```python
from build123d import *

# Parameters (mm, degrees)
SKETCH1_R           = 20
SKETCH1_R_2         = 10
BOSS_EXTRUDE1_DEPTH = 8
SKETCH2_R           = 18
SKETCH2_R_2         = 13
CUT_EXTRUDE1_DEPTH  = 5.5


with BuildPart() as part:
    # Sketch1 → Boss-Extrude1 (new body)
    with BuildSketch(Plane(origin=(0, 0, 0), x_dir=(1, 0, 0), z_dir=(0, 1, 0))):
        with Locations(Location((0, 0, 0), (0, 0, 270))):
            Circle(SKETCH1_R)
        with Locations(Location((0, 0, 0), (0, 0, 270))):
            Circle(SKETCH1_R_2, mode=Mode.SUBTRACT)
    extrude(amount=BOSS_EXTRUDE1_DEPTH)

    # Sketch2 → Cut-Extrude1 (cut)
    with BuildSketch(Plane(origin=(0, 8, 0), x_dir=(1, 0, 0), z_dir=(0, 1, 0))):
        with Locations(Location((0, 0, 0), (0, 0, 270))):
            Circle(SKETCH2_R)
        with Locations(Location((0, 0, 0), (0, 0, 270))):
            Circle(SKETCH2_R_2, mode=Mode.SUBTRACT)
    extrude(amount=-CUT_EXTRUDE1_DEPTH, mode=Mode.SUBTRACT)


solid = part.part
```
Check sheet for the modelled part. Datum: model origin and axes. Units: mm. A direction names the side the tool comes from. Give positions to 0.01 mm unless a question says otherwise; leave off trailing zeros. Order: outer loops, then holes, each group sorted by start corner. A loop starts at its lowest first (then second) coordinate and runs counter-clockwise, first axis right, second up. Notation, with made-up numbers: (40, 57.5) -> (55, 57.5) arc R16 cw to (55, 65.5) -> close; hole circle Ø8 at (74, 19.5). An arc over 180 degrees is marked (long way). Use CSV: the item, a comma, the result in double quotes. Start each with the question number.
1) Material ranges on line 1 (X direction, y = 6.85, z = 0); line 2 (Z direction, x = 7.5, y = 4); line 3 (X direction, y = 5.5, z = 12), recorded low to high. Write a range as from..to.
2) Sectioned sample at C-C, the plane y = 6.5. Record the boundary of the cut face in (x, z).
3) Sectioned sample at B-B, the plane z = 4.5. Record the boundary of the cut face in (x, y).
4) Sectioned sample at A-A, the plane x = 0. Record the boundary of the cut face in (y, z), plus the area to 3 significant figures.
5) Mould release check, pull along X, two halves, no side actions. Record for faces 3 (the face through (-9.76, 3.94, -2.17)), 4 (the face through (-19.524, 3.944, -4.336)), 5 (the face through (-8, 8, 7)): released by +X, released by -X, zero draft, split by the parting line, or undercut.
6) Set-up check for faces 1 (the face through (3, 8, -18)), 2 (the face through (-7.91, 5.288, -10.316)): record each of +Z, -Z, +X, -X, +Y, -Y from which the full face is reachable in a straight line by a thin tool's end or side.
7) Go/stop test with flat-tipped pins: P1, Ø2, axis at x = 6, z = 8.5, coming from the -Y side; P2, Ø3, axis at y = 3, z = -12.5, coming from the -X side. Record where each tip stops, or that it passes through.
8) Sectioned sample at D-D, the plane z = -10.5. Record the boundary of the cut face in (x, y), plus the area to 3 significant figures.
Recorded:
1,line 1,"-20..-18, -13..-10, 10..13, 18..20"
1,line 2,"-18.54..-16.36, -10.62..-6.61, 6.61..10.62, 16.36..18.54"
1,line 3,"-16..-13.42, -5..5, 13.42..16"
2,outline,"circle Ø40 at (0, 0); circle Ø26 at (0, 0); hole circle Ø36 at (0, 0); hole circle Ø20 at (0, 0)"
3,outline,"(-19.49, 0) -> (-8.93, 0) -> (-8.93, 8) -> (-12.2, 8) -> (-12.2, 2.5) -> (-17.43, 2.5) -> (-17.43, 8) -> (-19.49, 8) -> close; (8.93, 0) -> (19.49, 0) -> (19.49, 8) -> (17.43, 8) -> (17.43, 2.5) -> (12.2, 2.5) -> (12.2, 8) -> (8.93, 8) -> close"
4,outline,"(0, -20) -> (8, -20) -> (8, -18) -> (2.5, -18) -> (2.5, -13) -> (8, -13) -> (8, -10) -> (0, -10) -> close; (0, 10) -> (8, 10) -> (8, 13) -> (2.5, 13) -> (2.5, 18) -> (8, 18) -> (8, 20) -> (0, 20) -> close"
4,area,"105 mm2"
5,face 3,"undercut"
5,face 4,"split by the parting line"
5,face 5,"zero draft"
6,face 1,"+Z, -Z, +X, -X, +Y"
6,face 2,"+Y"
7,P1,"y = 0"
7,P2,"x = -16.7"
8,outline,"(-17.02, 0) -> (17.02, 0) -> (17.02, 8) -> (14.62, 8) -> (14.62, 2.5) -> (7.66, 2.5) -> (7.66, 8) -> (-7.66, 8) -> (-7.66, 2.5) -> (-14.62, 2.5) -> (-14.62, 8) -> (-17.02, 8) -> close"
8,area,"196 mm2"
